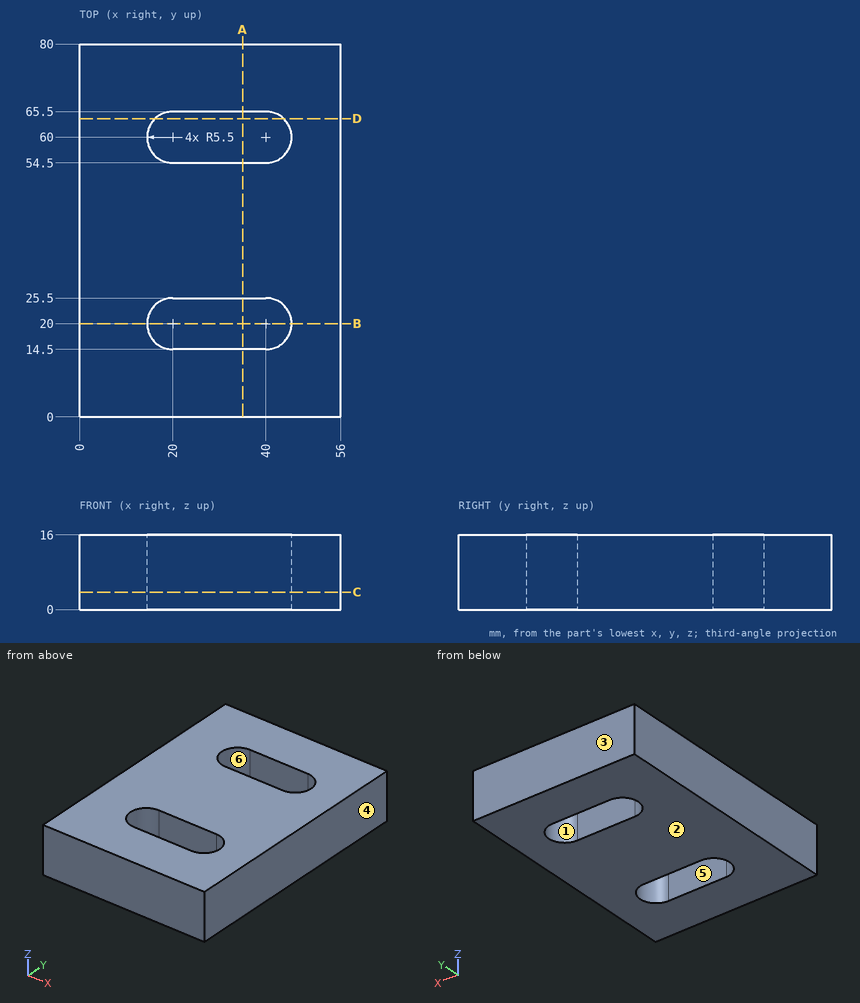
Geometry check sheet. Reference: drawing and pictorial views, mm from the part's lowest x, y, z. A direction names the side the tool comes from. Coordinates: 2 decimals unless noted, no trailing zeros. Order: outer loops, then holes, each group sorted by start corner. A loop starts at its lowest first (then second) coordinate and runs counter-clockwise, first axis right, second up. Notation, with made-up numbers: (32.5, -3) - (89.5, -3) arc R15 ccw to (89.5, 5) - close; hole circle Ø9 at (78, 17). An arc over 180 degrees is marked (long way). One line per item, written item: value.
(1) Access from +Z, -Z, +X, -X, +Y, -Y to the whole of each face (thin tool, end or side, straight path). Record for the marked faces 1 and 2.
Data:
face 1: +Z, -Z
face 2: -Z, +X, -X, +Y, -Y
(2) Thickness scan on probe 1 along Y at (x, z) = (29.5, 5.5); probe 2 along Y at (x, z) = (17.5, 9.5); probe 3 along X at (y, z) = (64.5, 1). Record the ranges inside material, lowest first. Write a range as from..to.
Data:
probe 1: y = 0..14.5, 25.5..54.5, 65.5..80
probe 2: y = 0..15.1, 24.9..55.1, 64.9..80
probe 3: x = 0..16.84, 43.16..56
(3) Sectioned sample at D-D (y = 64). Enter the section's corners in (x, z).
Data:
outline: (0, 0) - (16.23, 0) - (16.23, 16) - (0, 16) - close; (43.77, 0) - (56, 0) - (56, 16) - (43.77, 16) - close
(4) Sectioned sample at C-C (z = 3.75). Enter the section's corners in (x, y), and give its area (3 significant figures).
Data:
outline: (0, 0) - (56, 0) - (56, 80) - (0, 80) - close; hole (20, 14.5) - (40, 14.5) arc R5.5 ccw to (40, 25.5) - (20, 25.5) arc R5.5 ccw to start; hole (20, 54.5) - (40, 54.5) arc R5.5 ccw to (40, 65.5) - (20, 65.5) arc R5.5 ccw to start
area: 3,850 mm^2
(5) Sectioned sample at A-A (x = 35). Enter the section's corners in (y, z), and give its area (3 significant figures).
Data:
outline: (0, 0) - (14.5, 0) - (14.5, 16) - (0, 16) - close; (25.5, 0) - (54.5, 0) - (54.5, 16) - (25.5, 16) - close; (65.5, 0) - (80, 0) - (80, 16) - (65.5, 16) - close
area: 928 mm^2
(6) Release check for a two-part mould opening along Y. For the marked faces 3, 4, 5 and 6 record: +Y half, -Y half, draft (parallel to the pull), parting line (faces both ways), or undercut.
Data:
face 3: +Y half
face 4: draft
face 5: undercut
face 6: undercut
(7) Sectioned sample at B-B (y = 20). Enter the section's corners in (x, z), and give its area (3 significant figures).
Data:
outline: (0, 0) - (14.5, 0) - (14.5, 16) - (0, 16) - close; (45.5, 0) - (56, 0) - (56, 16) - (45.5, 16) - close
area: 400 mm^2
